Could you check a few things on this model? Use its own coordinates, in mm. Face numbers are marked on the shaded views. Round coordinates to 2 decimals unless told otherwise and drop trailing zeros. Write each loop counter-clockwise with the first axis right and the second up, starting at its lowest first coordinate (ties: lowest second). Pieces come first, ordered by that corner, then holes. Notation, with made-up numbers: (-2.75, 15.5) -> (43.25, 15.5) arc R23 ccw to (43.25, 28.5) -> close; hole circle Ø6 at (-22, -35.5). An arc over 180 degrees is marked (long way). Answer in a Markdown table with one row per item. Add a question column.
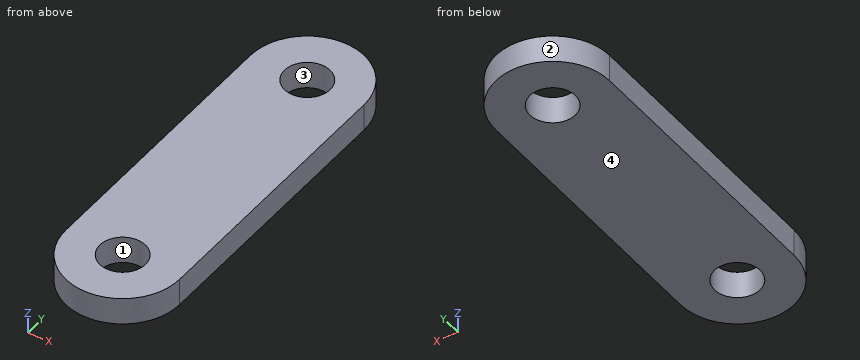
```python
from build123d import *

# Parameters (mm, degrees)
SKETCH1_R           = 5
BOSS_EXTRUDE1_DEPTH = 3


with BuildPart() as part:
    # Sketch1 → Boss-Extrude1 (new, symmetric)
    with BuildSketch(Plane.XY):
        with BuildLine():
            Line((-12.5, 0), (-12.5, 60))
            ThreePointArc((-12.5, 60), (0, 72.5), (12.5, 60))
            Line((12.5, 60), (12.5, 0))
            ThreePointArc((12.5, 0), (0, -12.5), (-12.5, 0))
        make_face()
        Circle(SKETCH1_R, mode=Mode.SUBTRACT)
        with Locations((0, 60)):
            Circle(SKETCH1_R, mode=Mode.SUBTRACT)
    extrude(amount=BOSS_EXTRUDE1_DEPTH, both=True)


solid = part.part
```
(1) I need wall thicknesses on L1, parallel to Y at x = 0, z = 1.7; L2, parallel to Y at x = 3, z = 2.65; L3, parallel to X at y = 62, z = 0.3. Which ranges of each line are inside material? Lowest first, please.
(2) Suppose I cut it at A-A, the plane x = 0. Please give me the cut outline in (y, z), then the cut area to 3 significant figures.
(3) For P1, Ø3, axis at x = 0.5, y = 3.5, coming from the +Z side; P2, Ø1.5, axis at x = 9.5, z = -1, coming from the +Y side, each with a flat end and sliding along its axis, tell me the tip position at first contact or that it passes through.
(4) Suppose I cut it at D-D, the plane y = 3.5. Please give me the cut outline in (x, z), then the cut area to 3 significant figures.
(5) Suppose I cut it at C-C, the plane z = -2.15. Please give me the cut outline in (x, y), then the cut area to 3 significant figures.
(6) If we mould it in two halves opening along Y, with no side actions, what happens to the marked faces 1, 2, 3 and 4? For each: pulls with the +Y half, pulls with the -Y half, needs draft (parallel to the pull), parting line crosses it, or undercut.
(7) Suppose I cut it at B-B, the plane y = 57. Please give me the cut outline in (x, z).
Response:
| question | item | result |
|---|---|---|
| 1 | L1 | -12.5 to -5, 5 to 55, 65 to 72.5 |
| 1 | L2 | -12.13 to -4, 4 to 56, 64 to 72.13 |
| 1 | L3 | -12.34 to -4.58, 4.58 to 12.34 |
| 2 | outline | (-12.5, -3) -> (-5, -3) -> (-5, 3) -> (-12.5, 3) -> close; (5, -3) -> (55, -3) -> (55, 3) -> (5, 3) -> close; (65, -3) -> (72.5, -3) -> (72.5, 3) -> (65, 3) -> close |
| 2 | area | 390 mm² |
| 3 | P1 | z = 3 |
| 3 | P2 | y = 68.93 |
| 4 | outline | (-12.5, -3) -> (-3.57, -3) -> (-3.57, 3) -> (-12.5, 3) -> close; (3.57, -3) -> (12.5, -3) -> (12.5, 3) -> (3.57, 3) -> close |
| 4 | area | 107 mm² |
| 5 | outline | (-12.5, 0) arc R12.5 ccw to (12.5, 0) -> (12.5, 60) arc R12.5 ccw to (-12.5, 60) -> close; hole circle Ø10 at (0, 0); hole circle Ø10 at (0, 60) |
| 5 | area | 1,830 mm² |
| 6 | face 1 | undercut |
| 6 | face 2 | pulls with the +Y half |
| 6 | face 3 | undercut |
| 6 | face 4 | needs draft |
| 7 | outline | (-12.5, -3) -> (-4, -3) -> (-4, 3) -> (-12.5, 3) -> close; (4, -3) -> (12.5, -3) -> (12.5, 3) -> (4, 3) -> close |
